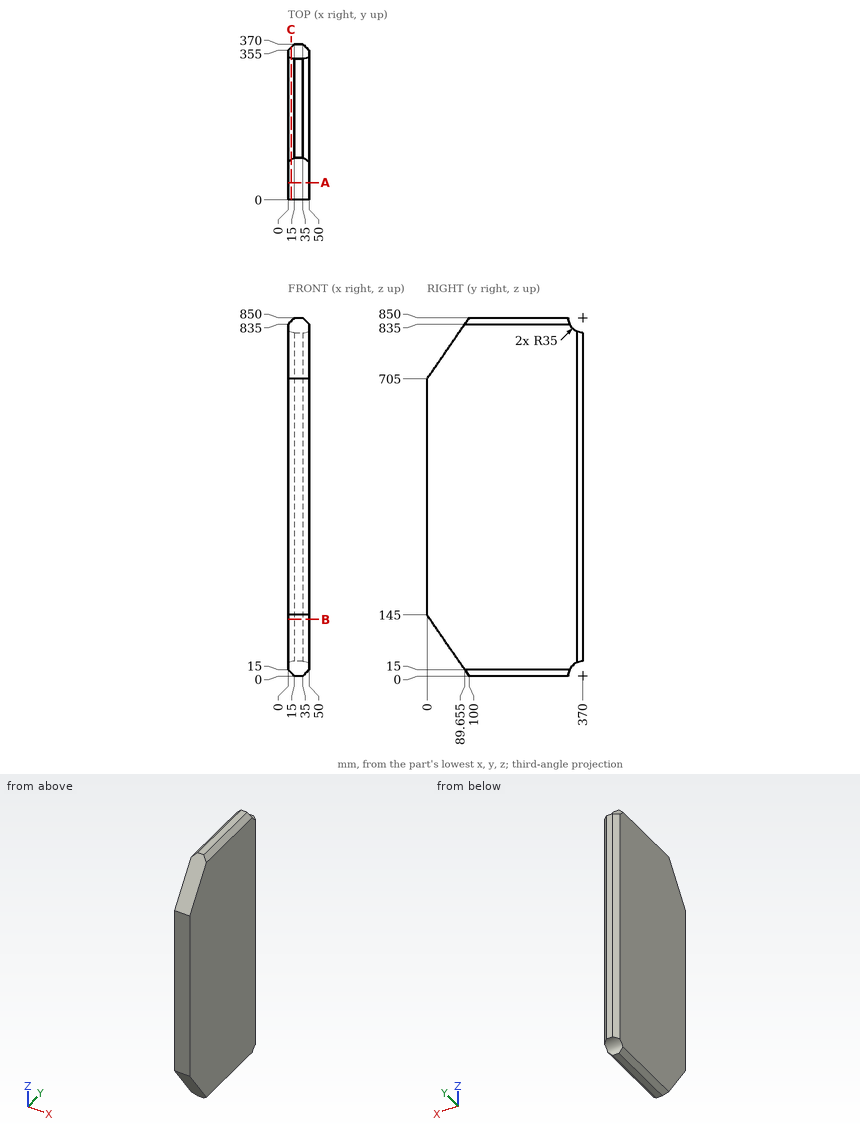
Answer from the drawing. Dimensions are ordinates in mm from the lowest x, y and z of the part. Round coordinates to 2 decimals unless told otherwise and drop trailing zeros. Order: outer loops, then holes, each group sorted by start corner. A loop starts at its lowest first (then second) coordinate and runs counter-clockwise, first axis right, second up. Notation, with made-up numbers: (67.25, -1.5) - (99.25, -1.5) arc R17 ccw to (99.25, 8.5) - close; hole circle Ø4 at (10.5, 73.5). An arc over 180 degrees is marked (long way). Put each result on its own line as item: value. Start each with the question number.
(1) Find section A-A (y = 41). Give the vertices of the cut face in (x, z), plus the area to 3 significant figures.
(2) Straight lines are drawn through the part: probe 1 along Z at (x, y) = (47, 194); probe 2 along Y at (x, z) = (13.5, 793); probe 3 along Z at (x, y) = (34, 69). For each, find the intervals that lie inside material, in ascending order. Write a range as from..to.
(3) Find section B-B (z = 134.5). Give the vertices of the cut face in (x, y).
(4) Given P1, Ø5, axis at x = 31, y = 89.5, coming from the -Z side, flat-ended and moving along its own axis, determine where the tip first touches the part or whether it passes through.
(5) Find section C-C (x = 7.5). Give the vertices of the cut face in (y, z).
Reply:
1. outline: (0, 85.55) - (50, 85.55) - (50, 764.45) - (0, 764.45) - close
1. area: 33,900 mm^2
2. probe 1: 12..838
2. probe 2: 60.69..368.5
2. probe 3: 44.95..805.05
3. outline: (0, 7.24) - (50, 7.24) - (50, 355) - (35, 370) - (15, 370) - (0, 355) - close
4. P1: z = 11.6
5. outline: (0, 145) - (94.83, 7.5) - (335.81, 7.5) arc R35 cw to (362.5, 34.19) - (362.5, 815.81) arc R35 cw to (335.81, 842.5) - (94.83, 842.5) - (0, 705) - close
